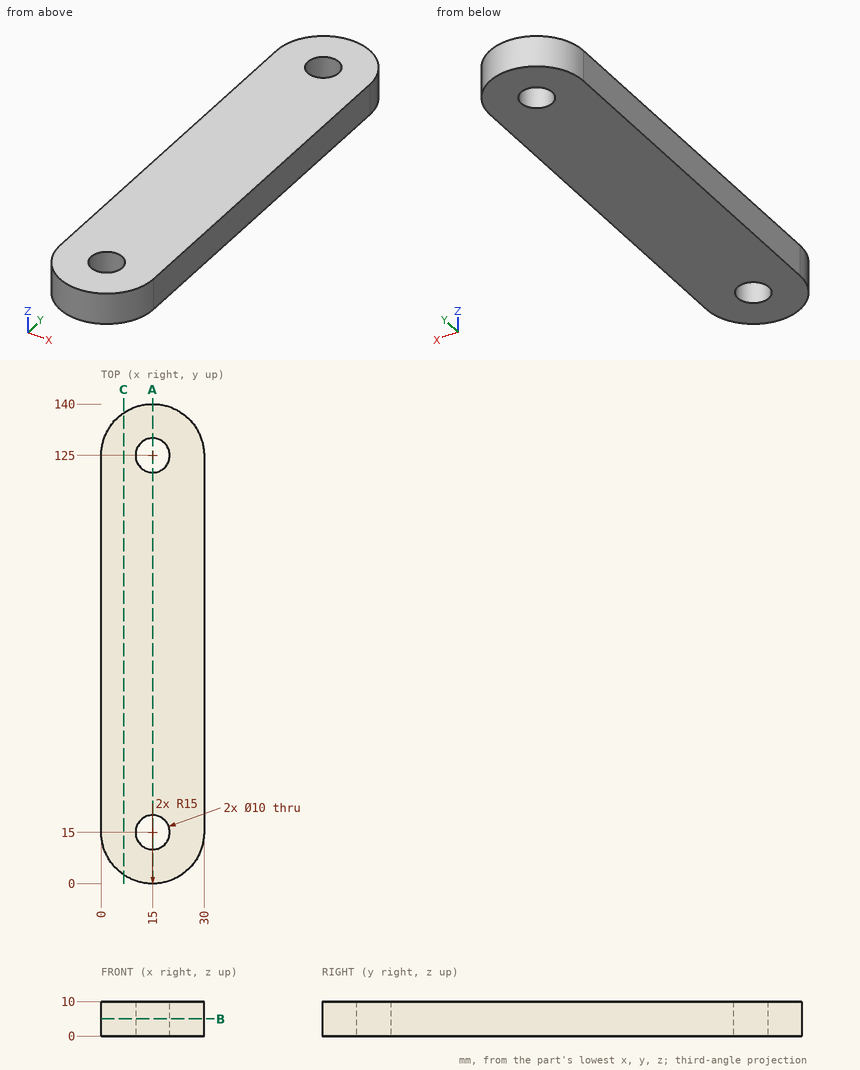
Job drawing, mm, ordinate dimensions from the low corner. One solid piece. Give positions to 0.01 mm unless a question says otherwise; leave off trailing zeros. Write each loop counter-clockwise with the first axis right and the second up, starting at its lowest first coordinate (ties: lowest second). Pieces come first, ordered by that corner, then holes. Notation, with made-up numbers: M 37,68.5 L 76,68.5 A11 ccw 76,84.5 Z; hole C 50,-15 d6. An arc over 180 degrees is marked long. One line per item, written item: value. Start each with the question number.
Q1. Saw through at C-C, the plane x = 6.5. Write the cut outline in (y, z).
Q2. Drop flat-ended pins along their axis: pin 1 Ø5 at (x, z) = (8.5, 8.5) entering from -Y; pin 2 Ø4 at (x, z) = (6, 3) entering from +Y. Give the stop position or say it passes through.
Q3. Probe probe 1 along Y at (x, z) = (15, 8); probe 2 along Y at (x, z) = (16.5, 5.5); probe 3 along X at (y, z) = (18, 8.5). List the from-to ranges inside material, lowest first. Write a range as [from, to].
Q4. Saw through at A-A, the plane x = 15. Write the cut outline in (y, z).
Q5. Saw through at B-B, the plane z = 5. Write the cut outline in (x, y).
Output values:
1. outline: M 2.64,0 L 137.36,0 L 137.36,10 L 2.64,10 Z
2. pin 1: stops at y = 0.54
2. pin 2: stops at y = 138.27
3. probe 1: y = [0, 10], [20, 120], [130, 140]
3. probe 2: y = [0.08, 10.23], [19.77, 120.23], [129.77, 139.92]
3. probe 3: x = [0, 11], [19, 30]
4. outline: M 0,0 L 10,0 L 10,10 L 0,10 Z; M 20,0 L 120,0 L 120,10 L 20,10 Z; M 130,0 L 140,0 L 140,10 L 130,10 Z
5. outline: M 0,15 A15 ccw 30,15 L 30,125 A15 ccw 0,125 Z; hole C 15,15 d10; hole C 15,125 d10
